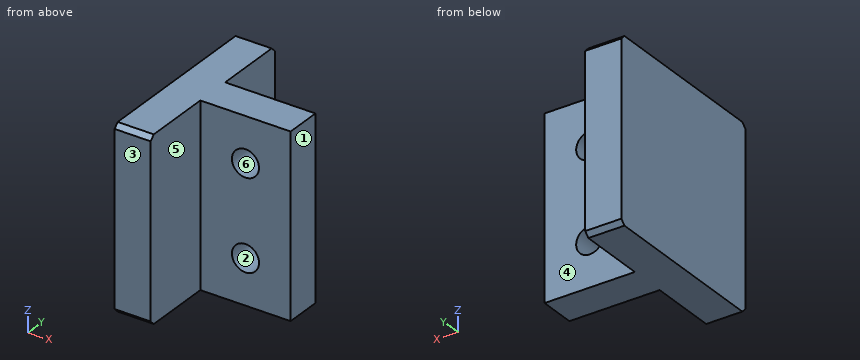
```python
from build123d import *

# Parameters (mm, degrees)
SKETCH1_W               = 8
SKETCH1_H               = 40
BOSS_EXTRUDE1_DEPTH     = 40
CHAMFER1_SIZE           = 1
SKETCH2_W               = 20
SKETCH2_H               = 8
BOSS_EXTRUDE2_DEPTH     = 40
CUT_EXTRUDE1_DEPTH      = 55.405882035
CUT_EXTRUDE1_DEPTH_BACK = 55.405882035
SKETCH4_R               = 3


with BuildPart() as part:
    # Sketch1 → Boss-Extrude1 (new body)
    with BuildSketch(Plane(origin=(0, 0, 0), x_dir=(1, 0, 0), z_dir=(0, 1, 0))):
        with Locations((4, -20)):
            Rectangle(SKETCH1_W, SKETCH1_H)
    extrude(amount=BOSS_EXTRUDE1_DEPTH)

    # Chamfer1
    chamfer1_edges = [part.edges().sort_by_distance(p)[0] for p in [
        (4, 40, 0),
        (4, 0, 0),
        (4, 0, 40),
        (4, 40, 40),
    ]]
    chamfer(chamfer1_edges, length=CHAMFER1_SIZE)

    # Sketch2 → Boss-Extrude2 (add)
    with BuildSketch(Plane.XY.offset(40)):
        with Locations((18, 20)):
            Rectangle(SKETCH2_W, SKETCH2_H)
    extrude(amount=-BOSS_EXTRUDE2_DEPTH)

    # Sketch4 → Cut-Extrude1 (cut, two sides: drawn at the far end of the back side and taken through both)
    with BuildSketch(Plane(origin=(0, 24, 0), x_dir=(1, 0, 0), z_dir=(0, 1, 0)).offset(-CUT_EXTRUDE1_DEPTH_BACK)):
        with Locations(Location((18, -30, 0), (0, 0, 180))):
            Circle(SKETCH4_R)
        with Locations(Location((18, -10, 0), (0, 0, 180))):
            Circle(SKETCH4_R)
    extrude(amount=CUT_EXTRUDE1_DEPTH + CUT_EXTRUDE1_DEPTH_BACK, mode=Mode.SUBTRACT)


solid = part.part
```
Source: CAD feature listing. Evaluate the final solid. Frame: model axes, mm. Face numbers are marked on the shaded views. A direction names the side the tool comes from. Round coordinates to 2 decimals unless told otherwise and drop trailing zeros. Loops run counter-clockwise (first coordinate to the right, second up) from the corner with the lowest first, then second, coordinate; pieces in that order, holes last. Notation, with made-up numbers: M 51.5,-28 L 96.5,-28 A24 cw 96.5,9 Z; hole C 88,6 d5. An arc over 180 degrees is marked long. Put each result on its own line as item: value.
(1) Access query for the marked faces 4, 5 and 6. Directions: +Z, -Z, +X, -X, +Y, -Y. A direction counts if a zero-diameter tool reaches every point of the face in a straight line with its end or side. Return the directions, or none.
Solutions:
face 4: +Z, -Z, +X, +Y
face 5: +Z, -Z, +X, -Y
face 6: +Y, -Y
(2) Pull-direction query (X, two-part tool) for the marked faces 1, 2 and 3; classes: released by +X, released by -X, zero draft, split by the parting line, or undercut.
Solutions:
face 1: released by +X
face 2: undercut
face 3: zero draft
(3) Ray query, line 1 (Z direction, x = 18, y = 22.5); line 2 (X direction, y = 20.25, z = 30); line 3 (Y direction, x = 15.25, z = 27). Return the intervals inside material, ascending. Write a range as [from, to].
Solutions:
line 1: [0, 7], [13, 27], [33, 40]
line 2: [0, 15], [21, 28]
line 3: [16, 24]
(4) Section B-B, the plane x = 18. Return loops of the section in (y, z), and give its area (3 significant figures).
Solutions:
outline: M 16,0 L 24,0 L 24,7 L 16,7 Z; M 16,13 L 24,13 L 24,27 L 16,27 Z; M 16,33 L 24,33 L 24,40 L 16,40 Z
area: 224 mm²
(5) Section A-A, the plane z = 30. Return loops of the section in (x, y).
Solutions:
outline: M 0,0 L 8,0 L 8,16 L 15,16 L 15,24 L 8,24 L 8,40 L 0,40 Z; M 21,16 L 28,16 L 28,24 L 21,24 Z
(6) Section C-C, the plane y = 21. Return loops of the section in (x, z), and give its area (3 significant figures).
Solutions:
outline: M 0,0 L 28,0 L 28,40 L 0,40 Z; hole C 18,10 d6; hole C 18,30 d6
area: 1,060 mm²
(7) Section D-D, the plane z = 37.5. Return loops of the section in (x, y).
Solutions:
outline: M 0,0 L 8,0 L 8,16 L 28,16 L 28,24 L 8,24 L 8,40 L 0,40 Z
(8) First-contact query: pin 1 (1 mm diameter, centred on y = 28.5, z = 9.5, fed in from +X); pin 2 (3 mm diameter, centred on x = 22, z = 10, fed in from +Y); pin 3 (3 mm diameter, centred on x = 15, z = 12.5, fed in from -Y). Flat tips, straight axial feed; report the tip coordinate or a pass-through.
Solutions:
pin 1: x = 8
pin 2: y = 24
pin 3: y = 16
